The listing builds one solid part. Answer for the finished solid, in the listing's coordinates (mm). Face numbers are marked on the shaded views. Give positions to 0.01 mm unless a question says otherwise; leave off trailing zeros. Order: outer loops, then holes, each group sorted by start corner. A loop starts at its lowest first (then second) coordinate and runs counter-clockwise, first axis right, second up. Notation, with made-up numbers: (79, 77) - (111, 77) arc R29 ccw to (111, 101) - close; hole circle Ø8 at (13, -15.5). An arc over 180 degrees is marked (long way). Answer as a JSON object with one key per item and string values. Group by question number.
Q1. Consider line 1 (Y direction, x = 0, z = -45); line 2 (Y direction, x = 0, z = 30.35); line 3 (Z direction, x = 65.5, y = 23.5). Determine where each line is inside the solid, lowest interval first.
Q2. Given pin 1 (3 mm diameter, centred on y = 35.5, z = 19, fed in from +X); pin 2 (4 mm diameter, centred on x = -41, y = -39, fed in from +Z); pin 3 (12 mm diameter, centred on y = 42.5, z = -35.5, fed in from +X); pin 4 (3 mm diameter, centred on x = -3, y = 72.5, fed in from -Z), each flat-ended and moving along its own axis, determine where each tip first touches the part or whether it passes through.
Q3. A cutting plane is placed at A-A, the plane z = -2. Give the vertices of the cut face in (x, y).
Q4. The mould has two halves that part along Y. Classify the marked faces 1 and 2: released by +Y, released by -Y, zero draft, split by the parting line, or undercut.
from build123d import *

# Parameters (mm, degrees)
SKETCH1_R                = 75
BOSS_EXTRUDE1_DEPTH      = 8
BOSS_EXTRUDE2_DEPTH      = 28
BOSS_EXTRUDE2_DEPTH_BACK = 56
SKETCH2_R                = 67.5
SKETCH3_R                = 60
CUT_EXTRUDE1_DEPTH       = 160
SKETCH4_W                = 5.197670867
SKETCH4_H                = 3.2
CHAMFER1_SIZE            = 1
SKETCH5_W                = 60
SKETCH5_H                = 150
CUT_EXTRUDE2_DEPTH       = 72
SKETCH6_R                = 8
CUT_EXTRUDE3_DEPTH       = 3


with BuildPart() as part:
    # Sketch1 → Boss-Extrude1 (new body)
    with BuildSketch(Plane.XY):
        Circle(SKETCH1_R)
    extrude(amount=BOSS_EXTRUDE1_DEPTH)

    # Sketch2 → Boss-Extrude2 (add, two sides: drawn at the far end of the back side and taken through both)
    with BuildSketch(Plane.XY.offset(8).offset(-BOSS_EXTRUDE2_DEPTH_BACK)):
        Circle(SKETCH2_R)
    extrude(amount=BOSS_EXTRUDE2_DEPTH + BOSS_EXTRUDE2_DEPTH_BACK)

    # Sketch3 → Cut-Extrude1 (cut)
    with BuildSketch(Plane.XY.offset(36)):
        Circle(SKETCH3_R)
    extrude(amount=-CUT_EXTRUDE1_DEPTH, mode=Mode.SUBTRACT)

    # Sketch4 → Cut-Revolve1 (revolve, cut)
    with BuildSketch(Plane(origin=(0, 0, 0), x_dir=(1, 0, 0), z_dir=(0, 1, 0)), mode=Mode.PRIVATE) as cut_revolve1_sk:
        with Locations((-59.401164567, -30.6)):
            Rectangle(SKETCH4_W, SKETCH4_H)
        with Locations((-59.401164567, 42.6)):
            Rectangle(SKETCH4_W, SKETCH4_H)
    revolve(cut_revolve1_sk.sketch.rotate(Axis((0, 0, -49.990530135), (0, 0, 1)), 180), axis=Axis((0, 0, -49.990530135), (0, 0, 1)), mode=Mode.SUBTRACT)

    # Chamfer1
    chamfer1_edges = [part.edges().sort_by_distance(p)[0] for p in [
        (-60, 0, -48),
        (-60, 0, 36),
        (-75, 0, 0),
        (-75, 0, 8),
        (-67.5, 0, -48),
        (-67.5, 0, 36),
    ]]
    chamfer(chamfer1_edges, length=CHAMFER1_SIZE)

    # Sketch5 → Cut-Extrude2 (cut)
    with BuildSketch(Plane(origin=(0, 0, 0), x_dir=(-1, 0, 0), z_dir=(0, 0, -1))):
        with Locations((-102, 0)):
            Rectangle(SKETCH5_W, SKETCH5_H)
        with Locations((102, 0)):
            Rectangle(SKETCH5_W, SKETCH5_H)
    extrude(amount=-CUT_EXTRUDE2_DEPTH, mode=Mode.SUBTRACT)

    # Sketch6 → Cut-Extrude3 (cut)
    with BuildSketch(Plane.XY):
        with Locations((0, 79.5)):
            Circle(SKETCH6_R)
        with Locations((0, -79.5)):
            Circle(SKETCH6_R)
    extrude(amount=CUT_EXTRUDE3_DEPTH, mode=Mode.SUBTRACT)


solid = part.part
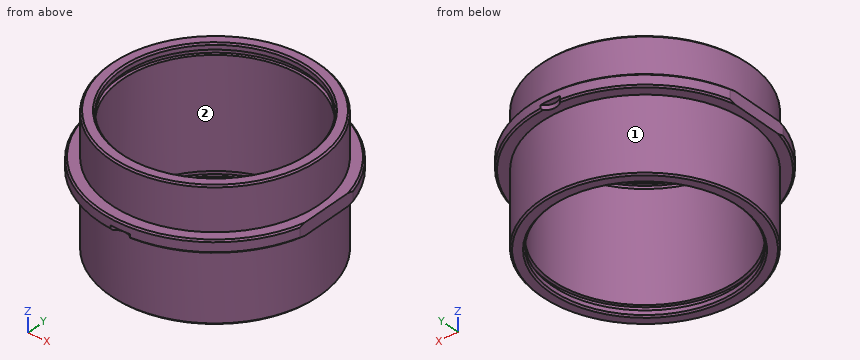
Reply:
{
 "1": {"line 1": "y = -67.5 to -60, 60 to 67.5", "line 2": "y = -67.5 to -62, 62 to 67.5", "line 3": "z = 0 to 8"},
 "2": {"pin 1": "stops at x = 58.31", "pin 2": "passes through", "pin 3": "stops at x = 56.78", "pin 4": "stops at z = 0"},
 "3": {"outline": "circle Ø135 at (0, 0); hole circle Ø120 at (0, 0)"},
 "4": {"face 1": "split by the parting line", "face 2": "undercut"}
}
